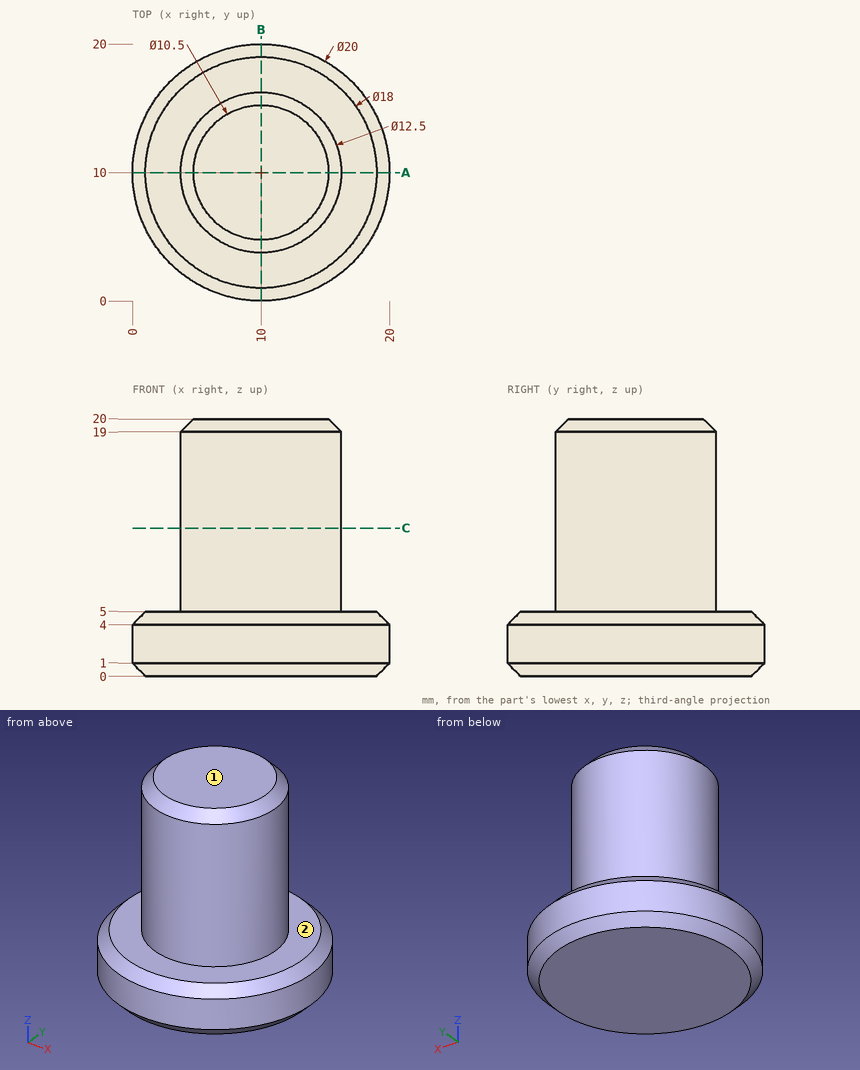
Verification items for this drawing (mm, ordinates from the low corner). A direction names the side the tool comes from. Round coordinates to 2 decimals unless told otherwise and drop trailing zeros. Order: outer loops, then holes, each group sorted by start corner. A loop starts at its lowest first (then second) coordinate and runs counter-clockwise, first axis right, second up. Notation, with made-up numbers: (58, -13) - (115, -13) arc R17 cw to (115, -3) - close; hole circle Ø6 at (-25, -7). An arc over 180 degrees is marked (long way). Answer as CSV lines item,"result". Start each with the question number.
1) Section check A-A (y = 10). Record the cut outline in (x, z).
2) Tool access check on the marked faces 1 and 2. Record the directions out of +Z, -Z, +X, -X, +Y, -Y that give a thin tool (end or side, any length) a straight path to the whole face; none if there is none.
3) Depth check by flat-ended pin: pin 1 (10 mm diameter, centred on y = 14.5, z = 7, fed in from +X); pin 2 (10 mm diameter, centred on x = 3, z = 9.5, fed in from +Y); pin 3 (6 mm diameter, centred on x = 10, z = 12, fed in from -Y); pin 4 (8 mm diameter, centred on x = 9.5, z = 7, fed in from -Y). Enter the tip coordinate at first touch or a pass-through.
4) Section check C-C (z = 11.5). Record the cut outline in (x, y).
5) Scan lines: probe 1 along Z at (x, y) = (2.75, 14.75); probe 2 along X at (y, z) = (9.75, 8.75) (3 decimals); probe 3 along Y at (x, z) = (6, 16.25). Record each from-to range of solid material in increasing order.
Determined:
1,outline,"(0, 1) - (1, 0) - (19, 0) - (20, 1) - (20, 4) - (19, 5) - (16.25, 5) - (16.25, 19) - (15.25, 20) - (4.75, 20) - (3.75, 19) - (3.75, 5) - (1, 5) - (0, 4) - close"
2,face 1,"+Z, +X, -X, +Y, -Y"
2,face 2,"+Z"
3,pin 1,"x = 19.99"
3,pin 2,"y = 17.6"
3,pin 3,"y = 3.75"
3,pin 4,"y = 0"
4,outline,"circle Ø12.5 at (10, 10)"
5,probe 1,"0 to 5"
5,probe 2,"3.755 to 16.245"
5,probe 3,"5.2 to 14.8"
